Job drawing, mm, ordinate dimensions from the low corner. One solid piece. Round coordinates to 2 decimals unless told otherwise and drop trailing zeros. Write each loop counter-clockwise with the first axis right and the second up, starting at its lowest first coordinate (ties: lowest second). Pieces come first, ordered by that corner, then holes.
1) Saw through at B-B on x = 7. Write the cut outline in (y, z), and give its area (3 significant figures).
2) Saw through at C-C on z = 3.75. Count the separate pieces of the cut face and the enclosed holes in it, and give its area (3 significant figures).
3) Drill centre lines: L1, parallel to Y at x = 7, z = 6; L2, parallel to Y at x = 64, z = 4.5; L3, parallel to X at y = 74, z = 8.25. Where is each one in solid material? Low to high.
4) Saw through at A-A on y = 32.5. Write the cut outline in (x, z).
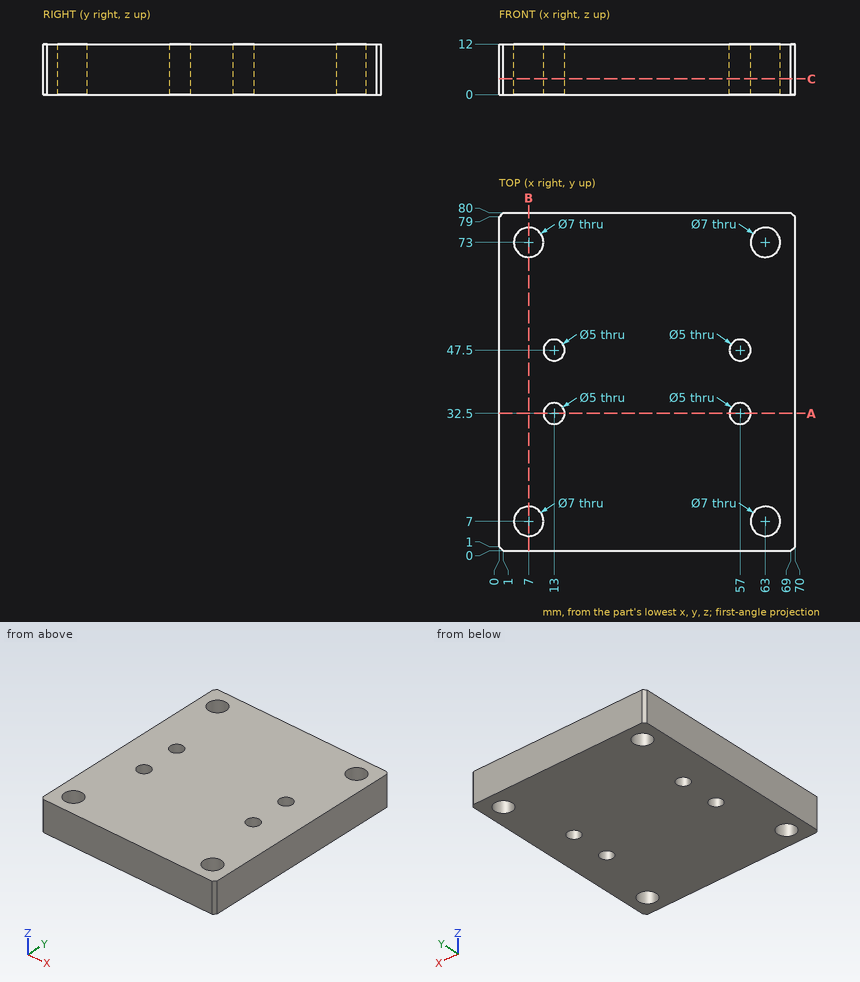
Completed:
1. outline: (0, 0) - (3.5, 0) - (3.5, 12) - (0, 12) - close; (10.5, 0) - (69.5, 0) - (69.5, 12) - (10.5, 12) - close; (76.5, 0) - (80, 0) - (80, 12) - (76.5, 12) - close
1. area: 792 mm2
2. separate pieces: 1
2. enclosed holes: 8
2. area: 5,370 mm2
3. L1: y = 0 to 3.5, 10.5 to 69.5, 76.5 to 80
3. L2: y = 0 to 3.65, 10.35 to 69.65, 76.35 to 80
3. L3: x = 0 to 3.65, 10.35 to 59.65, 66.35 to 70
4. outline: (0, 0) - (10.5, 0) - (10.5, 12) - (0, 12) - close; (15.5, 0) - (54.5, 0) - (54.5, 12) - (15.5, 12) - close; (59.5, 0) - (70, 0) - (70, 12) - (59.5, 12) - close
